Answer from the drawing. Dimensions are ordinates in mm from the lowest x, y and z of the part. A direction names the side the tool comes from. Give positions to 0.01 mm unless a question says otherwise; leave off trailing zeros. Order: outer loops, then holes, each group sorted by start corner. A loop starts at its lowest first (then second) coordinate and runs counter-clockwise, first axis right, second up. Notation, with made-up numbers: (-25.5, -35) -> (-4.5, -35) arc R16 cw to (-4.5, -21) -> close; hole circle Ø1 at (35, 50.25). An arc over 180 degrees is marked (long way). Write item = value, one per line. Start each with the question number.
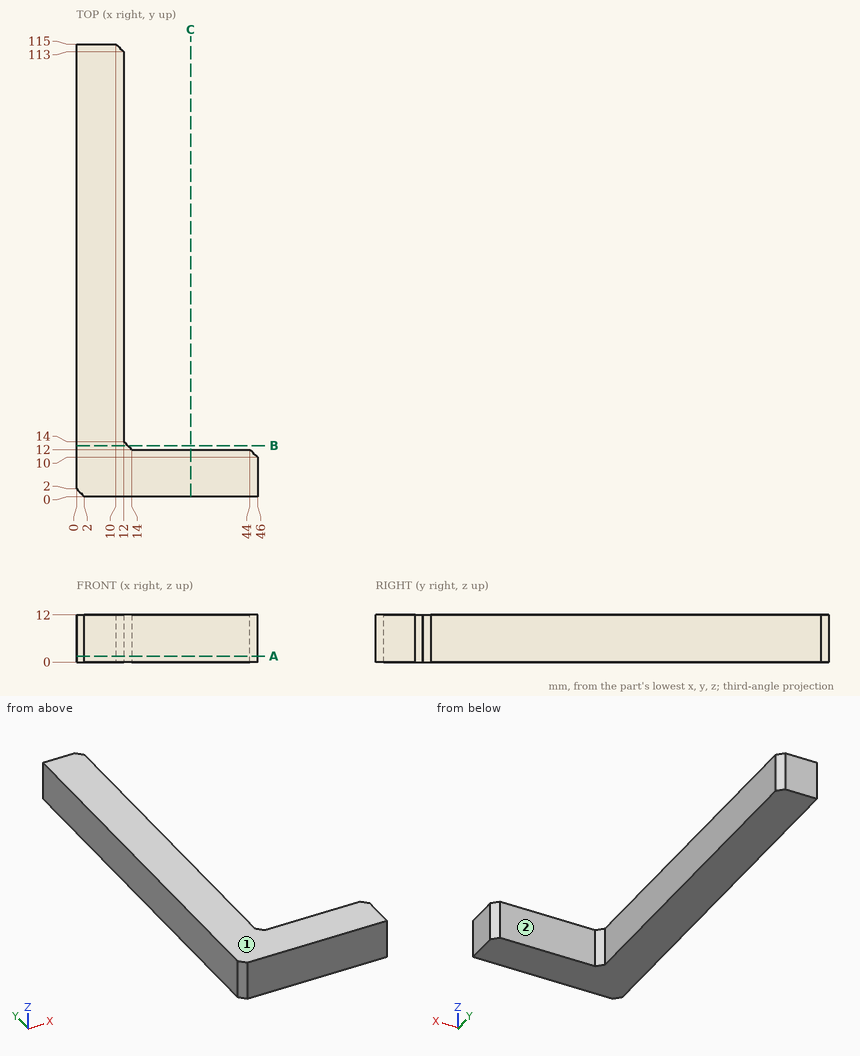
Item 1: Which of the six approach directions +Z, -Z, +X, -X, +Y, -Y give full straight-line access (tool end or side, diameter ignored) to the marked faces 1 and 2?
Item 2: A cutting plane is placed at B-B, the plane y = 13. Write down the section's boundary in (x, z).
Item 3: A cutting plane is placed at C-C, the plane x = 29. Write down the section's boundary in (y, z), plus the area to 3 significant figures.
Item 4: Consider L1, parallel to Y at x = 29.5, z = 10.75. Determine where the line is inside the solid, lowest interval first. Write a range as from..to.
Item 5: A cutting plane is placed at A-A, the plane z = 1.5. Write down the section's boundary in (x, y), plus the area to 3 significant figures.
Item 6: Flat-ended cylindrical pins translate along their axes: pin 1 (5 mm diameter, centred on y = 20, z = 3.5, fed in from +X); pin 2 (3 mm diameter, centred on x = 31, z = 2, fed in from +Y); pin 3 (1 mm diameter, centred on x = 13.5, y = 22, fed in from +Z). Find the tip coordinate at first contact, or state that the pin passes through.
Check values:
q1.face_1 = +Z, +X, -X, +Y, -Y
q1.face_2 = +Z, -Z, +X, +Y
q2.outline = (0, 0) -> (13, 0) -> (13, 12) -> (0, 12) -> close
q3.outline = (0, 0) -> (12, 0) -> (12, 12) -> (0, 12) -> close
q3.area = 144 mm^2
q4.L1 = 0..12
q5.outline = (0, 2) -> (2, 0) -> (46, 0) -> (46, 10) -> (44, 12) -> (14, 12) -> (12, 14) -> (12, 113) -> (10, 115) -> (0, 115) -> close
q5.area = 1,780 mm^2
q6.pin_1 = 12
q6.pin_2 = 12
q6.pin_3 = through
